For this review, take the finished solid that the model builds, in its own axes (mm). Face numbers are marked on the shaded views. Coordinates: 2 decimals unless noted, no trailing zeros. Write each loop counter-clockwise with the first axis right and the second up, starting at its lowest first coordinate (ties: lowest second). Pieces come first, ordered by that corner, then holes. Notation, with made-up numbers: M -30.75,-28.5 L 10.25,-28.5 A8 cw 10.25,-23.5 Z; hole C 65,-12.75 d4. An arc over 180 degrees is marked long. Return JSON: item names as keys, results as strings.
```python
from build123d import *

# Parameters (mm, degrees)
SKETCH1_W                                = 95
SKETCH1_H                                = 54
BOSS_EXTRUDE1_DEPTH                      = 10.05
SKETCH2_OUTSIDE_W                        = 118.948
SKETCH2_OUTSIDE_H                        = 77.948
SKETCH2_OUTSIDE_W_2                      = 93
SKETCH2_OUTSIDE_H_2                      = 52
CUT_EXTRUDE1_DEPTH                       = 1
CBORE_FOR_M3_PAN_HEAD_SCREW1_D           = 3.6
CBORE_FOR_M3_PAN_HEAD_SCREW1_CBORE_D     = 7
CBORE_FOR_M3_PAN_HEAD_SCREW1_CBORE_DEPTH = 2.4
CHAMFER1_SIZE                            = 1
CUT_EXTRUDE2_REACH                       = 111.736
SKETCH5_R                                = 8


with BuildPart() as part:
    # Sketch1 → Boss-Extrude1 (new body)
    with BuildSketch(Plane(origin=(0, 0, 0), x_dir=(1, 0, 0), z_dir=(0, 1, 0))):
        with Locations((47.5, 27)):
            Rectangle(SKETCH1_W, SKETCH1_H)
    extrude(amount=BOSS_EXTRUDE1_DEPTH)

    # Sketch2 outside → Cut-Extrude1 (cut)
    with BuildSketch(Plane(origin=(0, 10.05, 0), x_dir=(1, 0, 0), z_dir=(0, 1, 0))):
        with Locations((47.5, 27)):
            Rectangle(SKETCH2_OUTSIDE_W, SKETCH2_OUTSIDE_H)
        with Locations((47.5, 27)):
            Rectangle(SKETCH2_OUTSIDE_W_2, SKETCH2_OUTSIDE_H_2, mode=Mode.SUBTRACT)
    extrude(amount=-CUT_EXTRUDE1_DEPTH, mode=Mode.SUBTRACT)

    # CBORE for M3 Pan Head Screw1 (through all)
    with Locations(Plane(origin=(6, 10.05, -48), x_dir=(0, 0, 1), z_dir=(0, 1, 0))):
        with Locations((0, 0), (0, 83), (42, 83), (42, 0)):
            CounterBoreHole(CBORE_FOR_M3_PAN_HEAD_SCREW1_D / 2, CBORE_FOR_M3_PAN_HEAD_SCREW1_CBORE_D / 2, CBORE_FOR_M3_PAN_HEAD_SCREW1_CBORE_DEPTH)

    # Chamfer1
    chamfer1_edges = [part.edges().sort_by_distance(p)[0] for p in [
        (6, 10.05, -9.5),
        (89, 10.05, -9.5),
        (89, 10.05, -51.5),
        (6, 10.05, -51.5),
    ]]
    chamfer(chamfer1_edges, length=CHAMFER1_SIZE)

    # Sketch5 → Cut-Extrude2 (cut, up to next)
    with BuildSketch(Plane(origin=(0, 10.05, 0), x_dir=(1, 0, 0), z_dir=(0, 1, 0)), mode=Mode.PRIVATE) as cut_extrude2_sk1:
        with Locations(Location((47.5, 42, 0), (0, 0, 270))):
            Circle(SKETCH5_R)
    cut_extrude2_tool1 = extrude(cut_extrude2_sk1.sketch, amount=-CUT_EXTRUDE2_REACH, mode=Mode.PRIVATE) & part.part
    # Sketch5 → Cut-Extrude2 (cut, up to next)
    with BuildSketch(Plane(origin=(0, 10.05, 0), x_dir=(1, 0, 0), z_dir=(0, 1, 0)), mode=Mode.PRIVATE) as cut_extrude2_sk2:
        with Locations(Location((47.5, 12, 0), (0, 0, 270))):
            Circle(SKETCH5_R)
    cut_extrude2_tool2 = extrude(cut_extrude2_sk2.sketch, amount=-CUT_EXTRUDE2_REACH, mode=Mode.PRIVATE) & part.part
    add(cut_extrude2_tool1.solids().sort_by_distance((47.5, 10.05, -42))[0], mode=Mode.SUBTRACT)
    add(cut_extrude2_tool2.solids().sort_by_distance((47.5, 10.05, -12))[0], mode=Mode.SUBTRACT)


solid = part.part
```
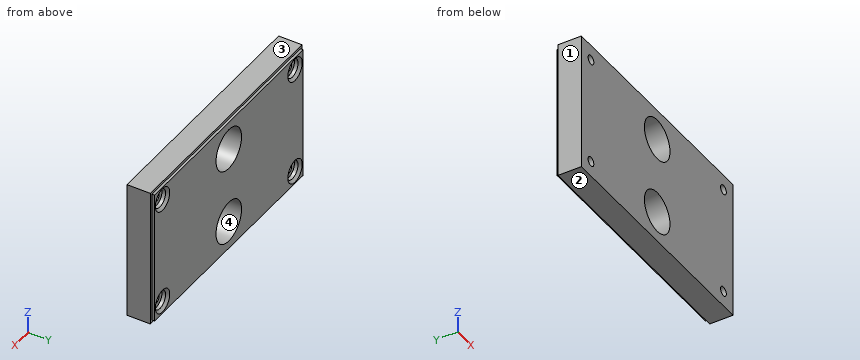
1. We need section B-B (y = 3.25). State the section outline as (x, z) points, plus the area to 3 significant figures.
Checks:
{"outline": "M 0,-54 L 95,-54 L 95,0 L 0,0 Z; hole C 6,-48 d3.6; hole C 6,-6 d3.6; hole C 47.5,-42 d16; hole C 47.5,-12 d16; hole C 89,-48 d3.6; hole C 89,-6 d3.6", "area": "4,690 mm2"}
2. We need section A-A (x = 47.5). State the section outline as (y, z) points.
Checks:
{"outline": "M 0,-54 L 9.05,-54 L 9.05,-53 L 10.05,-53 L 10.05,-50 L 0,-50 Z; M 0,-34 L 10.05,-34 L 10.05,-20 L 0,-20 Z; M 0,-4 L 10.05,-4 L 10.05,-1 L 9.05,-1 L 9.05,0 L 0,0 Z"}
3. We need section C-C (z = -42). State the section outline as (x, y) points.
Checks:
{"outline": "M 0,0 L 39.5,0 L 39.5,10.05 L 1,10.05 L 1,9.05 L 0,9.05 Z; M 55.5,0 L 95,0 L 95,9.05 L 94,9.05 L 94,10.05 L 55.5,10.05 Z"}
4. Clearance check with flat-ended pins moving along their axes: pin 1 Ø0.5 at (y, z) = (9.5, -30.5) entering from +X; pin 2 Ø3 at (x, z) = (89, -6) entering from +Y; pin 3 Ø5.5 at (x, z) = (88.5, -48.5) entering from +Y; pin 4 Ø5.5 at (x, z) = (6.5, -47) entering from +Y. State where each tip first meets the part, or that it passes through.
Checks:
{"pin 1": "x = 94", "pin 2": "through", "pin 3": "y = 7.65", "pin 4": "y = 9.42"}
5. Wall thickness on L1, parallel to Z at x = 89, y = 7.5; L2, parallel to X at y = 8.7, z = -6; L3, parallel to Z at x = 50, y = 6.5: over which ranges is each line inside the solid? List them lowest first. Write a range as from..to.
Checks:
{"L1": "-54..-49.8, -46.2..-7.8, -4.2..0", "L2": "0..2.5, 9.5..42.21, 52.79..85.5, 92.5..95", "L3": "-54..-49.6, -34.4..-19.6, -4.4..0"}
6. We need section D-D (x = 89). State the section outline as (y, z) points.
Checks:
{"outline": "M 0,-54 L 9.05,-54 L 9.05,-53 L 10.05,-53 L 10.05,-52.5 L 9.05,-51.5 L 7.65,-51.5 L 7.65,-49.8 L 0,-49.8 Z; M 0,-46.2 L 7.65,-46.2 L 7.65,-44.5 L 9.05,-44.5 L 10.05,-43.5 L 10.05,-10.5 L 9.05,-9.5 L 7.65,-9.5 L 7.65,-7.8 L 0,-7.8 Z; M 0,-4.2 L 7.65,-4.2 L 7.65,-2.5 L 9.05,-2.5 L 10.05,-1.5 L 10.05,-1 L 9.05,-1 L 9.05,0 L 0,0 Z"}
7. Draft analysis for pull direction Z (two halves, no side actions). For the marked faces 1, 2, 3 and 4, state which applies: +Z half, -Z half, draft (parallel to the pull), parting line (faces both ways), or undercut.
Checks:
{"face 1": "draft", "face 2": "-Z half", "face 3": "+Z half", "face 4": "undercut"}
